The figure shows three views and two pictorial views of one solid part (mm, origin at its lowest corner). Answer the questions. Round coordinates to 2 decimals unless told otherwise and drop trailing zeros. Loops run counter-clockwise (first coordinate to the right, second up) from the corner with the lowest first, then second, coordinate; pieces in that order, holes last. Notation, with made-up numbers: (-31.75, 9) -> (0.25, 9) arc R26 cw to (0.25, 25) -> close; hole circle Ø8 at (0, 82). An arc over 180 degrees is marked (long way). Put each result on its own line as item: value.
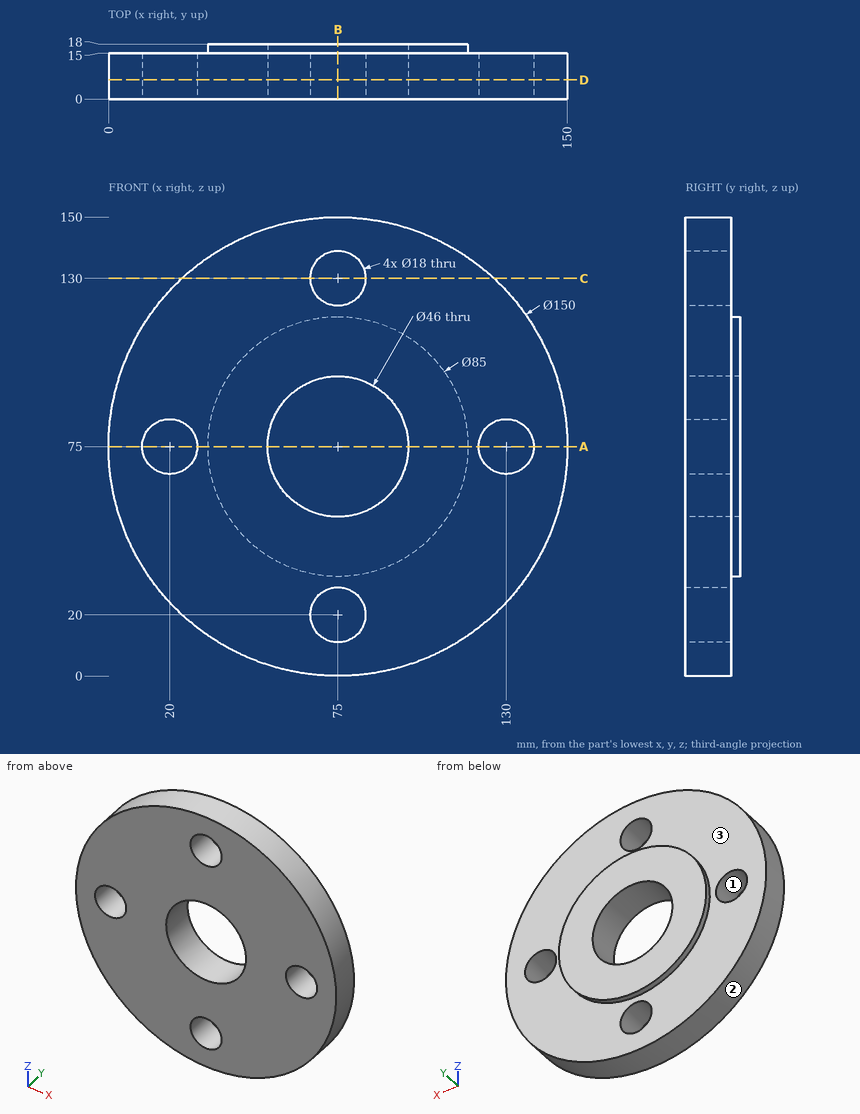
Item 1: The part is cut by section B-B (x = 75). Determine the outline of the cut face in (y, z).
Derived:
outline: (0, 0) -> (15, 0) -> (15, 11) -> (0, 11) -> close; (0, 29) -> (15, 29) -> (15, 32.5) -> (18, 32.5) -> (18, 52) -> (0, 52) -> close; (0, 98) -> (18, 98) -> (18, 117.5) -> (15, 117.5) -> (15, 121) -> (0, 121) -> close; (0, 139) -> (15, 139) -> (15, 150) -> (0, 150) -> close
Item 2: Flat-ended cylindrical pins translate along their axes: pin 1 Ø4 at (y, z) = (9.5, 25.5) entering from -X; pin 2 Ø8 at (x, y) = (42, 12.5) entering from +Z; pin 3 Ø1.5 at (x, z) = (28.5, 24) entering from +Y; pin 4 Ø6 at (x, z) = (55.5, 106.5) entering from -Y. Find the tip coordinate at first contact, or state that the pin passes through.
Derived:
pin 1: stops at x = 16.96
pin 2: stops at z = 144.17
pin 3: stops at y = 15
pin 4: stops at y = 0
Item 3: The part is cut by section A-A (z = 75). Determine the outline of the cut face in (x, y), then the cut area to 3 significant figures.
Derived:
outline: (0, 0) -> (11, 0) -> (11, 15) -> (0, 15) -> close; (29, 0) -> (52, 0) -> (52, 18) -> (32.5, 18) -> (32.5, 15) -> (29, 15) -> close; (98, 0) -> (121, 0) -> (121, 15) -> (117.5, 15) -> (117.5, 18) -> (98, 18) -> close; (139, 0) -> (150, 0) -> (150, 15) -> (139, 15) -> close
area: 1,140 mm^2
Item 4: For a pull along Z with two mould halves and no side action, classify the marked faces 1, 2 and 3 as pulls with the +Z half, pulls with the -Z half, needs draft (parallel to the pull), parting line crosses it, or undercut.
Derived:
face 1: undercut
face 2: parting line crosses it
face 3: needs draft
Item 5: Find the intervals of material crossed by line 1 along X through (y, z) = (10.5, 75); line 2 along Z through (x, y) = (74, 7.75); line 3 along Y through (x, z) = (140.5, 57.5), in increasing order.
Derived:
line 1: x = 0 to 11, 29 to 52, 98 to 121, 139 to 150
line 2: z = 0.01 to 11.06, 28.94 to 52.02, 97.98 to 121.06, 138.94 to 149.99
line 3: y = 0 to 15
Item 6: The part is cut by section C-C (z = 130). Determine the outline of the cut face in (x, y).
Derived:
outline: (24.01, 0) -> (66, 0) -> (66, 15) -> (24.01, 15) -> close; (84, 0) -> (125.99, 0) -> (125.99, 15) -> (84, 15) -> close
Item 7: The part is cut by section D-D (y = 6.25). Determine the outline of the cut face in (x, z).
Derived:
outline: circle Ø150 at (75, 75); hole circle Ø18 at (20, 75); hole circle Ø46 at (75, 75); hole circle Ø18 at (75, 20); hole circle Ø18 at (75, 130); hole circle Ø18 at (130, 75)
